from build123d import *

# Parameters (mm, degrees)
SKETCH1_W           = 280
SKETCH1_H           = 415
SKETCH1_R           = 58
BOSS_EXTRUDE1_DEPTH = 25


with BuildPart() as part:
    # Sketch1 → Boss-Extrude1 (new body)
    with BuildSketch(Plane.XY):
        with Locations((140, -207.5)):
            Rectangle(SKETCH1_W, SKETCH1_H)
        with Locations((140, -355)):
            Circle(SKETCH1_R, mode=Mode.SUBTRACT)
    extrude(amount=BOSS_EXTRUDE1_DEPTH)


solid = part.part
Geometry: final body of the model. Coordinates: model frame, mm. Coordinates: 2 decimals unless noted, no trailing zeros. Order: outer loops, then holes, each group sorted by start corner. A loop starts at its lowest first (then second) coordinate and runs counter-clockwise, first axis right, second up.
(1) Section query B-B (x = 140). Return the cut outline in (y, z).
(2) First-contact query: pin 1 (3 mm diameter, centred on x = 101.5, z = 8, fed in from +Y). Flat tip, straight axial feed; report the tip coordinate or a pass-through.
(3) Draft query along Y for faces 1 (the face through (166.76, -406.46, 12.32)), 2 (the face through (138, 0, 12)), 3 (the face through (138, -415, 12)), 4 (the face through (0, -210, 12)). Return one class per face: pulls with the +Y half, pulls with the -Y half, needs draft (parallel to the pull), parting line crosses it, or undercut.
(4) Section query A-A (y = -355). Return the cut outline in (x, z).
(5) Material intervals for probe 1 along Y at (x, z) = (140, 8); probe 2 along Y at (x, z) = (100.5, 1.5); probe 3 along X at (y, z) = (-305, 5.25), sorted ascending.
Solution:
1. outline: (-415, 0) - (-413, 0) - (-413, 25) - (-415, 25) - close; (-297, 0) - (0, 0) - (0, 25) - (-297, 25) - close
2. pin 1: stops at y = 0
3. face 1: undercut
3. face 2: pulls with the +Y half
3. face 3: pulls with the -Y half
3. face 4: needs draft
4. outline: (0, 0) - (82, 0) - (82, 25) - (0, 25) - close; (198, 0) - (280, 0) - (280, 25) - (198, 25) - close
5. probe 1: y = -415 to -413, -297 to 0
5. probe 2: y = -415 to -397.47, -312.53 to 0
5. probe 3: x = 0 to 110.61, 169.39 to 280
